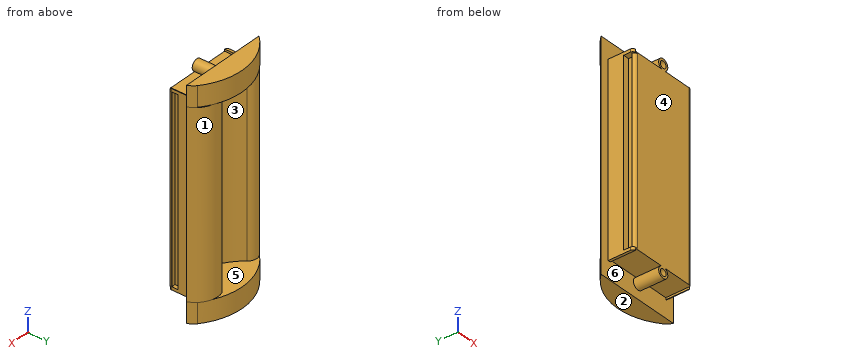
from build123d import *

# Parameters (mm, degrees)
EXTRUDE_1_DEPTH      = 45
EXTRUDE_2_DEPTH      = 10
CUT_EXTRUDE_11_DEPTH = 12.5
FILLET_1_R           = 1.5
SKETCH_4_R           = 1.7
CUT_EXTRUDE_12_DEPTH = 11.25


with BuildPart() as part:
    # 草图1 → 凸台-拉伸1 (new, symmetric)
    with BuildSketch(Plane.XY):
        with BuildLine():
            Line((-15.5, 0), (15.5, 0))
            ThreePointArc((15.5, 0), (16.560660172, 0.439339828), (17, 1.5))
            Line((17, 1.5), (17, 1.6))
            Line((17, 1.6), (15, 1.6))
            Line((15, 1.6), (15, 4.8))
            Line((15, 4.8), (17, 4.8))
            Line((17, 4.8), (17, 12.5))
            Line((17, 12.5), (21.25, 12.5))
            ThreePointArc((21.25, 12.5), (15.900063146, 18.351194202), (8.005834372, 19.085666803))
            ThreePointArc((8.005834372, 19.085666803), (7.659690231, 18.472905768), (8.269164703, 18.121007034))
            ThreePointArc((8.269164703, 18.121007034), (13.386035944, 17.124613538), (15.791887335, 12.5))
            ThreePointArc((15.791887335, 12.5), (12.736961816, 4.997664438), (5.127858316, 2.219328112))
            ThreePointArc((5.127858316, 2.219328112), (-5.972198102, 5.342922516), (-14.872141684, 12.674982166))
            ThreePointArc((-14.872141684, 12.674982166), (-18.60669741, 14.511266303), (-22.25, 12.5))
            Line((-22.25, 12.5), (-18, 12.5))
            Line((-18, 12.5), (-18, 4.8))
            Line((-18, 4.8), (-15, 4.8))
            Line((-15, 4.8), (-15, 1.6))
            Line((-15, 1.6), (-17, 1.6))
            Line((-17, 1.6), (-17, 1.5))
            ThreePointArc((-17, 1.5), (-16.560660172, 0.439339828), (-15.5, 0))
        make_face()
    extrude(amount=EXTRUDE_1_DEPTH, both=True)

    # 草图2 → 凸台-拉伸2 (add)
    with BuildSketch(Plane.XY.offset(45)):
        with BuildLine():
            Line((-22.25, 12.5), (-18, 12.5))
            Line((-18, 12.5), (-18, 1.5))
            Line((-18, 1.5), (-18, 0))
            Line((-18, 0), (-16.5, 0))
            Line((-16.5, 0), (16.5, 0))
            Line((16.5, 0), (17, 0))
            Line((17, 0), (17, 1.5))
            Line((17, 1.5), (17, 12.5))
            Line((17, 12.5), (21.25, 12.5))
            ThreePointArc((21.25, 12.5), (20.28562135, 14.348675496), (18.853738793, 15.864373227))
            ThreePointArc((18.853738793, 15.864373227), (-2.367503819, 22.360156158), (-22.25, 12.5))
        make_face()
    extrude_2 = extrude(amount=EXTRUDE_2_DEPTH)

    # 镜向1: 凸台-拉伸2 across plane
    add(extrude_2.mirror(Plane.XY))

    # 草图3 → 切除-拉伸11 (cut)
    with BuildSketch(Plane.XZ):
        with BuildLine():
            Line((1.145643924, 45.5), (16.73, 45.5))
            Line((16.73, 45.5), (16.73, 46.5))
            Line((16.73, 46.5), (18, 46.5))
            Line((18, 46.5), (18, 55))
            Line((18, 55), (-18, 55))
            Line((-18, 55), (-18, 46.5))
            Line((-18, 46.5), (-16.73, 46.5))
            Line((-16.73, 46.5), (-16.73, 45.5))
            Line((-16.73, 45.5), (-1.145643924, 45.5))
            ThreePointArc((-1.145643924, 45.5), (0, 50.75), (1.145643924, 45.5))
        make_face()
        with BuildLine():
            Line((-18, -46.5), (-18, -55))
            Line((-18, -55), (18, -55))
            Line((18, -55), (18, -46.5))
            Line((18, -46.5), (16.73, -46.5))
            Line((16.73, -46.5), (16.73, -45.5))
            Line((16.73, -45.5), (1.145643924, -45.5))
            ThreePointArc((1.145643924, -45.5), (0, -50.75), (-1.145643924, -45.5))
            Line((-1.145643924, -45.5), (-16.73, -45.5))
            Line((-16.73, -45.5), (-16.73, -46.5))
            Line((-16.73, -46.5), (-18, -46.5))
        make_face()
    extrude(amount=-CUT_EXTRUDE_11_DEPTH, mode=Mode.SUBTRACT)

    # 圆角1
    fillet_1_edges = [part.edges().sort_by_distance(p)[0] for p in [
        (-18, 0, -45.75),
        (17, 0, -45.75),
        (17, 0, 45.75),
        (-18, 0, 45.75),
    ]]
    fillet(fillet_1_edges, radius=FILLET_1_R)

    # 草图4 → 切除-拉伸12 (cut)
    with BuildSketch(Plane.XZ):
        with Locations(Location((0, 48, 0), (0, 0, 270))):
            Circle(SKETCH_4_R)
        with Locations(Location((0, -48, 0), (0, 0, 270))):
            Circle(SKETCH_4_R)
    extrude(amount=-CUT_EXTRUDE_12_DEPTH, mode=Mode.SUBTRACT)


solid = part.part
Verification items for the finished model (mm, model axes). Face numbers are marked on the shaded views. A direction names the side the tool comes from. Coordinates: 2 decimals unless noted, no trailing zeros. Order: outer loops, then holes, each group sorted by start corner. A loop starts at its lowest first (then second) coordinate and runs counter-clockwise, first axis right, second up. Notation, with made-up numbers: (10, 64) -> (68, 64) arc R23 ccw to (68, 98) -> close; hole circle Ø3 at (59, 16). An arc over 180 degrees is marked (long way). Use CSV: the item, a comma, the result in double quotes. Start each with the question number.
Q1. Thickness scan on line 1 along X through (y, z) = (3, 48); line 2 along Z through (x, y) = (1.5, 16.5); line 3 along Z through (x, y) = (6.5, 10.25). Record the ranges inside material, lowest first.
Q2. Draft check along X on the marked faces 1, 2 and 3. Enter one of: +X half, -X half, draft (parallel to the pull), parting line (faces both ways), or undercut.
Q3. Section check D-D, the plane y = 17. Record the cut outline in (x, z), and give its area (3 significant figures).
Q4. Depth check by flat-ended pin: P1, Ø6, axis at x = 9.5, z = 0.5, coming from the +Y side; P2, Ø4, axis at x = 12, y = 9, coming from the +Z side; P3, Ø5, axis at x = -5.5, z = 19.5, coming from the +Y side. Enter the tip coordinate at first touch or a pass-through.
Q5. Tool access check on the marked faces 4, 5 and 6. Record the directions out of +Z, -Z, +X, -X, +Y, -Y that give a thin tool (end or side, any length) a straight path to the whole face; none if there is none.
Q6. Section check C-C, the plane x = 0. Record the cut outline in (y, z), and give its area (3 significant figures).
Q7. Section check B-B, the plane z = 48. Record the cut outline in (x, y), and give its area (3 significant figures).
Q8. Section check A-A, the plane y = 6.5. Record the cut outline in (x, z).
Returned:
1,line 1,"x = -2.75 to -1.7, 1.7 to 2.75"
1,line 2,"z = -55 to -45, 45 to 55"
1,line 3,"z = -45.5 to -45, 45 to 45.5"
2,face 1,"parting line"
2,face 2,"draft"
2,face 3,"undercut"
3,outline,"(-17.18, -55) -> (17.34, -55) -> (17.34, -45) -> (17.99, -45) -> (17.99, 45) -> (17.34, 45) -> (17.34, 55) -> (-17.18, 55) -> (-17.18, 45) -> (13.55, 45) -> (13.55, -45) -> (-17.18, -45) -> close"
3,area,"1,090 mm^2"
4,P1,"stops at y = 19.5"
4,P2,"stops at z = 45.5"
4,P3,"stops at y = 6.51"
5,face 4,"+Z, -Z, +X, -X, -Y"
5,face 5,"none"
5,face 6,"-Y"
6,outline,"(0, -50.75) -> (12.5, -50.75) -> (12.5, -55) -> (22.46, -55) -> (22.46, -45) -> (3.05, -45) -> (3.05, 45) -> (22.46, 45) -> (22.46, 55) -> (12.5, 55) -> (12.5, 50.75) -> (0, 50.75) -> (0, 49.7) -> (11.25, 49.7) -> (11.25, 46.3) -> (0, 46.3) -> (0, -46.3) -> (11.25, -46.3) -> (11.25, -49.7) -> (0, -49.7) -> close"
6,area,"541 mm^2"
7,outline,"(-22.25, 12.5) -> (-2.75, 12.5) -> (-2.75, 0) -> (-1.7, 0) -> (-1.7, 11.25) -> (1.7, 11.25) -> (1.7, 0) -> (2.75, 0) -> (2.75, 12.5) -> (21.25, 12.5) arc R7.57 ccw to (18.85, 15.86) arc R30.01 ccw to start"
7,area,"337 mm^2"
8,outline,"(-18, -46.5) -> (-16.73, -46.5) -> (-16.73, -45.5) -> (-1.15, -45.5) arc R2.75 ccw (long way) to (1.15, -45.5) -> (16.73, -45.5) -> (16.73, -46.5) -> (17, -46.5) -> (17, 46.5) -> (16.73, 46.5) -> (16.73, 45.5) -> (1.15, 45.5) arc R2.75 ccw (long way) to (-1.15, 45.5) -> (-16.73, 45.5) -> (-16.73, 46.5) -> (-18, 46.5) -> close; hole (-7.98, -45) -> (14.02, -45) -> (14.02, 45) -> (-7.98, 45) -> close; hole circle Ø3.4 at (0, -48); hole circle Ø3.4 at (0, 48)"
